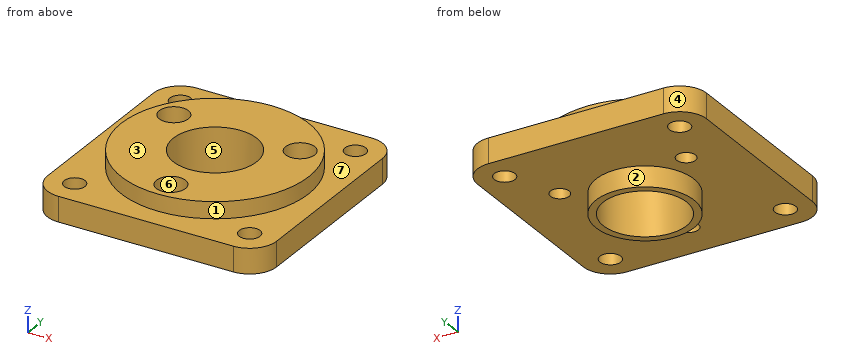
```python
from build123d import *

# Parameters (mm, degrees)
BOSS_EXTRUDE1_DEPTH = 12
SKETCH2_R           = 5
CUT_EXTRUDE1_DEPTH  = 50
SKETCH3_R           = 45
BOSS_EXTRUDE2_DEPTH = 8
SKETCH4_R           = 23.5
BOSS_EXTRUDE3_DEPTH = 9.8
SKETCH6_R           = 20
CUT_EXTRUDE2_DEPTH  = 80
SKETCH7_R           = 7
CUT_EXTRUDE3_DEPTH  = 9
SKETCH8_R           = 4.5
CUT_EXTRUDE4_DEPTH  = 801
CIRPATTERN1_COUNT   = 3


with BuildPart() as part:
    # Sketch1 → Boss-Extrude1 (new body)
    with BuildSketch(Plane.XY):
        with BuildLine():
            Line((-42, -55), (42, -55))
            ThreePointArc((42, -55), (51.192388155, -51.192388155), (55, -42))
            Line((55, -42), (55, 42))
            ThreePointArc((55, 42), (51.192388155, 51.192388155), (42, 55))
            Line((42, 55), (-42, 55))
            ThreePointArc((-42, 55), (-51.192388155, 51.192388155), (-55, 42))
            Line((-55, 42), (-55, -42))
            ThreePointArc((-55, -42), (-51.192388155, -51.192388155), (-42, -55))
        make_face()
    extrude(amount=BOSS_EXTRUDE1_DEPTH)

    # Sketch2 → Cut-Extrude1 (cut)
    with BuildSketch(Plane.XY.offset(12)):
        with Locations((42, 42)):
            Circle(SKETCH2_R)
        with Locations((42, -42)):
            Circle(SKETCH2_R)
        with Locations((-42, -42)):
            Circle(SKETCH2_R)
        with Locations((-42, 42)):
            Circle(SKETCH2_R)
    extrude(amount=-CUT_EXTRUDE1_DEPTH, mode=Mode.SUBTRACT)

    # Sketch3 → Boss-Extrude2 (add)
    with BuildSketch(Plane.XY.offset(12)):
        Circle(SKETCH3_R)
    extrude(amount=BOSS_EXTRUDE2_DEPTH)

    # Sketch4 → Boss-Extrude3 (add)
    with BuildSketch(Plane(origin=(0, 0, 0), x_dir=(-1, 0, 0), z_dir=(0, 0, -1))):
        with Locations(Location((0, 0, 0), (0, 0, 180))):
            Circle(SKETCH4_R)
    extrude(amount=BOSS_EXTRUDE3_DEPTH)

    # Sketch6 → Cut-Extrude2 (cut)
    with BuildSketch(Plane(origin=(0, 0, -9.8), x_dir=(-1, 0, 0), z_dir=(0, 0, -1))):
        Circle(SKETCH6_R)
    extrude(amount=-CUT_EXTRUDE2_DEPTH, mode=Mode.SUBTRACT)

    # Sketch7 → Cut-Extrude3 (cut)
    with BuildSketch(Plane.XY.offset(20)):
        with Locations((0, -35)):
            Circle(SKETCH7_R)
    cut_extrude3 = extrude(amount=-CUT_EXTRUDE3_DEPTH, mode=Mode.SUBTRACT)

    # Sketch8 → Cut-Extrude4 (cut)
    with BuildSketch(Plane.XY.offset(11)):
        with Locations((0, -35)):
            Circle(SKETCH8_R)
    cut_extrude4 = extrude(amount=-CUT_EXTRUDE4_DEPTH, mode=Mode.SUBTRACT)

    # CirPattern1: Cut-Extrude3, Cut-Extrude4 ×3 about axis
    cirpattern1_axis = Axis((0, 0, 0), (0, 0, 1))
    add([cut_extrude3.rotate(cirpattern1_axis, i * 360 / CIRPATTERN1_COUNT) for i in range(1, CIRPATTERN1_COUNT)], mode=Mode.SUBTRACT)
    add([cut_extrude4.rotate(cirpattern1_axis, i * 360 / CIRPATTERN1_COUNT) for i in range(1, CIRPATTERN1_COUNT)], mode=Mode.SUBTRACT)


solid = part.part
```
Read the model definition and answer for the solid it produces. Units are mm, in the model's axes. Face numbers are marked on the shaded views. A direction names the side the tool comes from. Coordinates: 2 decimals unless noted, no trailing zeros. Order: outer loops, then holes, each group sorted by start corner. A loop starts at its lowest first (then second) coordinate and runs counter-clockwise, first axis right, second up. Notation, with made-up numbers: (-16.5, 47) - (8.5, 47) arc R5 cw to (8.5, 55) - close; hole circle Ø11 at (51.25, -7). An arc over 180 degrees is marked (long way). Answer as a JSON object with one key per item and string values. Group by question number.
Item 1: The mould has two halves that part along Y. Classify the marked faces 4, 5, 6 and 7: +Y half, -Y half, draft (parallel to the pull), parting line (faces both ways), or undercut.
Item 2: A tool of negligible diameter and unlimited length cuts with its end or side. For the marked faces 1, 2 and 3, from which of +Z, -Z, +X, -X, +Y, -Y can it reach the whole face along a straight path? Write none if from no direction.
Item 3: Section D-D (x = 1) is taken. Give the vertices of the cut face in (y, z), plus the area to 3 significant figures.
Item 4: Consider probe 1 along X at (y, z) = (-42.5, 4.25); probe 2 along Y at (x, z) = (-42, 4.75); probe 3 along X at (y, z) = (-43, 5). Determine where each line is inside the solid, lowest interval first. Write a range as from..to.
Item 5: Section C-C (y = 17.5) is taken. State how many separate pieces and enclosed holes the cut face has, plus the area to 3 significant figures.
Item 6: Flat-ended cylindrical pins translate along their axes: P1, Ø15.5, axis at x = -28.5, y = 19, coming from the +Z side; P2, Ø8, axis at x = 42, y = -42, coming from the -Z side; P3, Ø22.5, axis at x = 0, y = -35, coming from the -Z side; P4, Ø4, axis at x = -35.5, z = 15, coming from the +Y side. Find the tip coordinate at first contact, or state that the pin passes through.
Item 7: Section B-B (x = -11) is taken. Give the vertices of the cut face in (y, z), plus the area to 3 significant figures.
Item 8: Section A-A (y = 0) is taken. Give the vertices of the cut face in (x, z).
Results are:
{
 "1": {"face 4": "+Y half", "face 5": "undercut", "face 6": "undercut", "face 7": "draft"},
 "2": {"face 1": "+Z", "face 2": "-Z", "face 3": "+Z, +X, -X, +Y, -Y"},
 "3": {"outline": "(-55, 0) - (-39.39, 0) - (-39.39, 11) - (-41.93, 11) - (-41.93, 20) - (-44.99, 20) - (-44.99, 12) - (-55, 12) - close; (-30.61, 0) - (-23.48, 0) - (-23.48, -9.8) - (-19.97, -9.8) - (-19.97, 20) - (-28.07, 20) - (-28.07, 11) - (-30.61, 11) - close; (19.97, -9.8) - (23.48, -9.8) - (23.48, 0) - (55, 0) - (55, 12) - (44.99, 12) - (44.99, 20) - (19.97, 20) - close", "area": "1,090 mm^2"},
 "4": {"probe 1": "x = -54.99..-46.97, -37.03..37.03, 46.97..54.99", "probe 2": "y = -55..-47, -37..37, 47..55", "probe 3": "x = -54.96..-46.9, -37.1..37.1, 46.9..54.96"},
 "5": {"separate pieces": "4", "enclosed holes": "0", "area": "1,260 mm^2"},
 "6": {"P1": "stops at z = 20", "P2": "passes through", "P3": "stops at z = 0", "P4": "stops at y = 30.05"},
 "7": {"outline": "(-55, 0) - (-20.77, 0) - (-20.77, -9.8) - (-16.7, -9.8) - (-16.7, 20) - (-43.63, 20) - (-43.63, 12) - (-55, 12) - close; (16.7, -9.8) - (20.77, -9.8) - (20.77, 0) - (55, 0) - (55, 12) - (43.63, 12) - (43.63, 20) - (16.7, 20) - close", "area": "1,430 mm^2"},
 "8": {"outline": "(-55, 0) - (-23.5, 0) - (-23.5, -9.8) - (-20, -9.8) - (-20, 20) - (-45, 20) - (-45, 12) - (-55, 12) - close; (20, -9.8) - (23.5, -9.8) - (23.5, 0) - (55, 0) - (55, 12) - (45, 12) - (45, 20) - (20, 20) - close"}
}
